Answer from the drawing. Dimensions are ordinates in mm from the lowest x, y and z of the part. Round coordinates to 2 decimals unless told otherwise and drop trailing zeros. Loops run counter-clockwise (first coordinate to the right, second up) from the corner with the lowest first, then second, coordinate; pieces in that order, holes last. Notation, with made-up numbers: M 41,-29.75 L 56,-29.75 A23 ccw 56,0.25 Z; hole C 39.25,80 d8. An arc over 180 degrees is marked long. Answer as CSV lines item,"result".
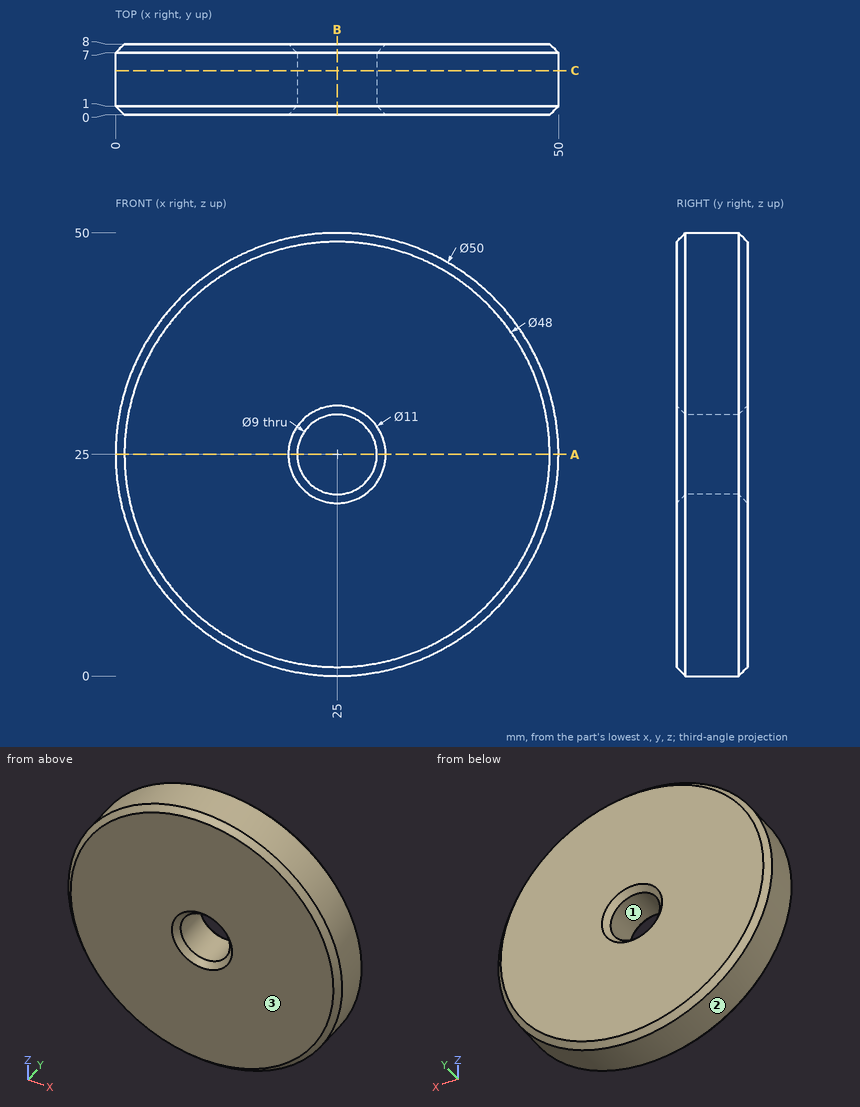
1) Straight lines are drawn through the part: line 1 (X direction, y = 3.6, z = 25); line 2 (Z direction, x = 21.5, y = 3); line 3 (X direction, y = 7.25, z = 25.5). For each, find the intervals that lie inside material, in ascending order.
Evaluation:
line 1,"x = 0 to 20.5, 29.5 to 50"
line 2,"z = 0.25 to 22.17, 27.83 to 49.75"
line 3,"x = 0.26 to 20.28, 29.72 to 49.74"
2) Find section B-B, the plane x = 25. Give the vertices of the cut face in (y, z), then the cut area to 3 significant figures.
Evaluation:
outline,"M 0,1 L 1,0 L 7,0 L 8,1 L 8,19.5 L 7,20.5 L 1,20.5 L 0,19.5 Z; M 0,30.5 L 1,29.5 L 7,29.5 L 8,30.5 L 8,49 L 7,50 L 1,50 L 0,49 Z"
area,"324 mm^2"
3) Determine the mould class of the marked faces 1, 2 and 3 for opening direction Z: released by +Z, released by -Z, zero draft, split by the parting line, or undercut.
Evaluation:
face 1,"undercut"
face 2,"split by the parting line"
face 3,"zero draft"
4) Each of these flat-tipped pins is pushed along its axis until it touches: P1, Ø1.5, axis at x = 31.5, y = 7, coming from the +Z side; P2, Ø1.5, axis at y = 1.5, z = 12.5, coming from the +X side; P3, Ø2, axis at x = 15, y = 2.5, coming from the +Z side. Where does it stop, or does it pass through?
Evaluation:
P1,"stops at z = 49.33"
P2,"stops at x = 47.07"
P3,"stops at z = 48.32"
5) Find section C-C, the plane y = 5. Give the vertices of the cut face in (x, z).
Evaluation:
outline,"C 25,25 d50; hole C 25,25 d9"
6) Find section A-A, the plane z = 25. Give the vertices of the cut face in (x, y).
Evaluation:
outline,"M 0,1 L 1,0 L 19.5,0 L 20.5,1 L 20.5,7 L 19.5,8 L 1,8 L 0,7 Z; M 29.5,1 L 30.5,0 L 49,0 L 50,1 L 50,7 L 49,8 L 30.5,8 L 29.5,7 Z"
